from build123d import *

# Parameters (mm, degrees)
SKETCH_1_W                = 80
SKETCH_1_H                = 70
EXTRUDE_1_DEPTH           = 12.5
SKETCH_3_W                = 80
SKETCH_3_H                = 66.5
CUT_EXTRUDE_1_DEPTH       = 2
HOLE_WIZARD_M5_1_D        = 4.2
HOLE_WIZARD_M6_1_D        = 5
CHAMFER_1_SIZE            = 2
HOLE_WIZARD_1_D           = 6.6
HOLE_WIZARD_1_DEPTH       = 25
HOLE_WIZARD_1_CBORE_D     = 11
HOLE_WIZARD_1_CBORE_DEPTH = 7


with BuildPart() as part:
    # 草图1 → 凸台-拉伸1 (new, symmetric)
    with BuildSketch(Plane(origin=(0, 0, 0), x_dir=(1, 0, 0), z_dir=(0, 1, 0))):
        Rectangle(SKETCH_1_W, SKETCH_1_H)
    extrude(amount=EXTRUDE_1_DEPTH, both=True)

    # 草图3 → 切除-拉伸1 (cut)
    with BuildSketch(Plane.XZ.offset(12.5)):
        with Locations((0, 1.75)):
            Rectangle(SKETCH_3_W, SKETCH_3_H)
    extrude(amount=-CUT_EXTRUDE_1_DEPTH, mode=Mode.SUBTRACT)

    # M5 螺纹孔1 (through all)
    with Locations(Plane(origin=(0, -10.5, 0), x_dir=(-1, 0, 0), z_dir=(0, -1, 0))):
        with Locations((20, 26.5), (-20, 26.5), (-20, -26.5), (20, -26.5)):
            Hole(HOLE_WIZARD_M5_1_D / 2)

    # M6 螺纹孔1 (through all)
    with Locations(Plane(origin=(0, -10.5, 0), x_dir=(-1, 0, 0), z_dir=(0, -1, 0))):
        with Locations((32.5, 22.5), (32.5, -22.5), (-32.5, 22.5), (-32.5, -22.5)):
            Hole(HOLE_WIZARD_M6_1_D / 2)

    # 倒角1
    chamfer_1_edges = [part.edges().sort_by_distance(p)[0] for p in [
        (-40, 0, -35),
        (40, 0, -35),
        (40, 1, 35),
        (-40, 1, 35),
    ]]
    chamfer(chamfer_1_edges, length=CHAMFER_1_SIZE)

    # 打孔尺寸(%根据)内六角花形圆柱头螺钉1
    with Locations(Plane(origin=(0, 12.5, 0), x_dir=(1, 0, 0), z_dir=(0, 1, 0))):
        with Locations((20, 26.5), (20, -26.5), (-20, -26.5), (-20, 26.5)):
            CounterBoreHole(HOLE_WIZARD_1_D / 2, HOLE_WIZARD_1_CBORE_D / 2, HOLE_WIZARD_1_CBORE_DEPTH, depth=HOLE_WIZARD_1_DEPTH)


solid = part.part
Could you check a few things on this model? Use its own coordinates, in mm. A direction names the side the tool comes from. Coordinates: 2 decimals unless noted, no trailing zeros. Loops run counter-clockwise (first coordinate to the right, second up) from the corner with the lowest first, then second, coordinate; pieces in that order, holes last.
1. For P1, Ø8.5, axis at x = 20, z = -26.5, coming from the -Y side; P2, Ø5.5, axis at x = 21.5, z = -28, coming from the +Y side; P3, Ø5.5, axis at x = -20, z = -26.5, coming from the +Y side; P4, Ø2, axis at x = 9.5, y = -12, coming from the +Z side, each with a flat end and sliding along its axis, tell me the tip position at first contact or that it passes through.
2. Imagine slicing it at A-A (x = -31). Please give me the cut outline in (y, z).
3. Imagine slicing it at D-D (x = 32.5). Please give me the cut outline in (y, z).
4. I need wall thicknesses on L1, parallel to Z at x = 20, y = -3.5; L2, parallel to Z at x = -32.5, y = -3; L3, parallel to X at y = -6.75, z = -26.5. Which ranges of each line are inside material? Lowest first, please.
5. Imagine slicing it at B-B (z = -26.5). Please give me the cut outline in (x, y).
6. Imagine slicing it at C-C (y = -1.75). Give the number of separate pieces and of enclosed holes in the cut face, and give its area (3 significant figures).
7. We'd pull the mould along X, two halves only. Please class faces 1 (the face through (-39, 0, -34)), 2 (the face through (-1, 1, 35)), 3 (the face through (-32.83, 1.16, -24.98)), 4 (the face through (39, 0, -34)): released by +X, released by -X, zero draft, split by the parting line, or undercut.
8. For faces 5 (the face through (16.95, -2.61, 27.76)), 6 (the face through (-20, 5.5, -23)), 7 (the face through (-1, -10.5, 2)), which set-ups out of +Z, -Z, +X, -X, +Y, -Y let a thin tool reach every point of the face, with its end or its side?
Computed values:
1. P1: stops at y = -10.5
1. P2: stops at y = 5.5
1. P3: passes through
1. P4: stops at z = -31.5
2. outline: (-12.5, -35) - (12.5, -35) - (12.5, -24.5) - (-10.5, -24.5) - (-10.5, -31.5) - (-12.5, -31.5) - close; (-10.5, -20.5) - (12.5, -20.5) - (12.5, 20.5) - (-10.5, 20.5) - close; (-10.5, 24.5) - (12.5, 24.5) - (12.5, 35) - (-10.5, 35) - close
3. outline: (-12.5, -35) - (12.5, -35) - (12.5, -25) - (-10.5, -25) - (-10.5, -31.5) - (-12.5, -31.5) - close; (-10.5, -20) - (12.5, -20) - (12.5, 20) - (-10.5, 20) - close; (-10.5, 25) - (12.5, 25) - (12.5, 35) - (-10.5, 35) - close
4. L1: z = -35 to -29.8, -23.2 to 23.2, 29.8 to 35
4. L2: z = -35 to -25, -20 to 20, 25 to 35
4. L3: x = -40 to -23.3, -16.7 to 16.7, 23.3 to 40
5. outline: (-40, -10.5) - (-23.3, -10.5) - (-23.3, 5.5) - (-25.5, 5.5) - (-25.5, 12.5) - (-40, 12.5) - close; (-16.7, -10.5) - (16.7, -10.5) - (16.7, 5.5) - (14.5, 5.5) - (14.5, 12.5) - (-14.5, 12.5) - (-14.5, 5.5) - (-16.7, 5.5) - close; (23.3, -10.5) - (40, -10.5) - (40, 12.5) - (25.5, 12.5) - (25.5, 5.5) - (23.3, 5.5) - close
6. separate pieces: 1
6. enclosed holes: 8
6. area: 5,380 mm2
7. face 1: released by -X
7. face 2: zero draft
7. face 3: undercut
7. face 4: released by +X
8. face 5: +Y, -Y
8. face 6: +Y
8. face 7: +Z, +X, -X, -Y
